```python
from build123d import *

# Parameters (mm, degrees)
BOSS_EXTRUDE1_DEPTH = 291
CUT_EXTRUDE1_REACH  = 325.544


with BuildPart() as part:
    # Sketch2 → Boss-Extrude1 (new, symmetric)
    with BuildSketch(Plane(origin=(0, 0, 0), x_dir=(1, 0, 0), z_dir=(0, 1, 0))):
        with BuildLine():
            Line((7.875, -1.525), (92.125, -1.525))
            ThreePointArc((92.125, -1.525), (97.693465902, 0.781534098), (100, 6.35))
            Line((100, 6.35), (100, 90.6))
            ThreePointArc((100, 90.6), (97.693465902, 96.168465902), (92.125, 98.475))
            Line((92.125, 98.475), (7.875, 98.475))
            ThreePointArc((7.875, 98.475), (2.306534098, 96.168465902), (0, 90.6))
            Line((0, 90.6), (0, 6.35))
            ThreePointArc((0, 6.35), (2.306534098, 0.781534098), (7.875, -1.525))
        make_face()
        with BuildLine():
            Line((12.6, 4.775), (87.4, 4.775))
            ThreePointArc((87.4, 4.775), (91.854772721, 6.620227279), (93.7, 11.075))
            Line((93.7, 11.075), (93.7, 85.875))
            ThreePointArc((93.7, 85.875), (91.854772721, 90.329772721), (87.4, 92.175))
            Line((87.4, 92.175), (12.6, 92.175))
            ThreePointArc((12.6, 92.175), (8.145227279, 90.329772721), (6.3, 85.875))
            Line((6.3, 85.875), (6.3, 11.075))
            ThreePointArc((6.3, 11.075), (8.145227279, 6.620227279), (12.6, 4.775))
        make_face(mode=Mode.SUBTRACT)
    extrude(amount=BOSS_EXTRUDE1_DEPTH, both=True)

    # Sketch4 → Cut-Extrude1 (cut, up to next)
    with BuildSketch(Plane.XY.offset(1.525), mode=Mode.PRIVATE) as cut_extrude1_sk1:
        Polygon((100, 291), (0, 268), (0, 291), align=None)
    cut_extrude1_tool1 = extrude(cut_extrude1_sk1.sketch, amount=-CUT_EXTRUDE1_REACH, mode=Mode.PRIVATE) & part.part
    # Sketch4 → Cut-Extrude1 (cut, up to next)
    with BuildSketch(Plane.XY.offset(1.525), mode=Mode.PRIVATE) as cut_extrude1_sk2:
        Polygon((0, -291), (100, -268), (100, -291), align=None)
    cut_extrude1_tool2 = extrude(cut_extrude1_sk2.sketch, amount=-CUT_EXTRUDE1_REACH, mode=Mode.PRIVATE) & part.part
    add(cut_extrude1_tool1.solids().sort_by_distance((33.333333, 283.333333, 1.525))[0], mode=Mode.SUBTRACT)
    add(cut_extrude1_tool2.solids().sort_by_distance((66.666667, -283.333333, 1.525))[0], mode=Mode.SUBTRACT)


solid = part.part
```
Source: CAD feature listing. Evaluate the final solid. Frame: model axes, mm. A direction names the side the tool comes from. Give positions to 0.01 mm unless a question says otherwise; leave off trailing zeros. Loops run counter-clockwise (first coordinate to the right, second up) from the corner with the lowest first, then second, coordinate; pieces in that order, holes last. Notation, with made-up numbers: M -29,-11 L -14,-11 A18 cw -14,13 Z; hole C -37,88.5 d8. An arc over 180 degrees is marked long. Put each result on its own line as item: value.
Q1. Section A-A (z = -53). Return the cut outline in (x, y).
Response values:
outline: M 0,-291 L 6.3,-289.55 L 6.3,269.45 L 0,268 Z; M 93.7,-269.45 L 100,-268 L 100,291 L 93.7,289.55 Z
Q2. Section B-B (y = 101.5). Return the cut outline in (x, z) (3 decimals).
Response values:
outline: M 0,-90.6 A7.875 ccw 7.875,-98.475 L 92.125,-98.475 A7.875 ccw 100,-90.6 L 100,-6.35 A7.875 ccw 92.125,1.525 L 7.875,1.525 A7.875 ccw 0,-6.35 Z; hole M 6.3,-85.875 A6.3 ccw 12.6,-92.175 L 87.4,-92.175 A6.3 ccw 93.7,-85.875 L 93.7,-11.075 A6.3 ccw 87.4,-4.775 L 12.6,-4.775 A6.3 ccw 6.3,-11.075 Z
Q3. Line query: probe 1 along X at (y, z) = (-73, -65.5); probe 2 along Z at (x, y) = (14, -204) (3 decimals); probe 3 along Z at (x, y) = (93, 211.5). Output: solid intervals per line, ascending. Write a range as [from, to].
Response values:
probe 1: x = [0, 6.3], [93.7, 100]
probe 2: z = [-98.475, -92.175], [-4.775, 1.525]
probe 3: z = [-98.43, -88.76], [-8.19, 1.48]
Q4. Mould query, pull axis X, two halves, no side actions, for faces 1 (the flat face through (6.3, -6, -49)), 2 (the flat face through (49.3, -279.66, -3.33)), 3 (the flat face through (49, 4, 1.525)), 4 (the flat face through (93.7, 14, -48)). Classes: released by +X, released by -X, zero draft, split by the parting line, or undercut.
Response values:
face 1: undercut
face 2: released by +X
face 3: zero draft
face 4: undercut
Q5. Section C-C (x = 57.5). Return the cut outline in (y, z) (3 decimals), and give its area (3 significant figures).
Response values:
outline: M -277.775,-98.475 L 281.225,-98.475 L 281.225,-92.175 L -277.775,-92.175 Z; M -277.775,-4.775 L 281.225,-4.775 L 281.225,1.525 L -277.775,1.525 Z
area: 7,040 mm²
Q6. Reachability of faces 5 (the flat face through (49, 4, -4.775)), 6 (the flat face through (51, 4, -98.475)) from +Z, -Z, +X, -X, +Y, -Y: full face, straight path, thin tool, end or side. Return the list, or none.
Response values:
face 5: +Y, -Y
face 6: -Z, +X, -X, +Y, -Y
